from build123d import *

# Parameters (mm, degrees)
SKETCH1_W                                    = 250
SKETCH1_H                                    = 50
BOSS_EXTRUDE1_DEPTH                          = 20
FILLET1_R                                    = 10
LPATTERN1_COUNT                              = 3
LPATTERN1_PITCH                              = 60
CBORE_FOR_M10_HEXAGON_SOCKET_HEAD_CA_2_COUNT = 2
CBORE_FOR_M10_HEXAGON_SOCKET_HEAD_CA_2_PITCH = 210


with BuildPart() as part:
    # Sketch1 → Boss-Extrude1 (new body)
    with BuildSketch(Plane.XY):
        with Locations((-50, 0)):
            Rectangle(SKETCH1_W, SKETCH1_H)
    extrude(amount=BOSS_EXTRUDE1_DEPTH)

    # Fillet1
    fillet1_edges = [part.edges().sort_by_distance(p)[0] for p in [
        (-175, 25, 10),
        (75, 25, 10),
        (75, -25, 10),
        (-175, -25, 10),
    ]]
    fillet(fillet1_edges, radius=FILLET1_R)

    # Sketch2 → CBORE for M8 Hexagon socket head cap screws1 (revolve, cut)
    with BuildSketch(Plane(origin=(10, 0, 20), x_dir=(0, -1, 0), z_dir=(1, 0, 0))):
        Polygon((0, 0), (0, 24.953872786), (4.5, 22.25), (4.5, 9), (7.5, 9), (7.5, 0), align=None)
    cbore_for_m8_hexagon_socket_head_cap_scr = revolve(axis=Axis((10, 0, 26.35), (0, 0, -1)), mode=Mode.SUBTRACT)

    # LPattern1: CBORE for M8 Hexagon socket head cap screws1 ×3
    with Locations(*[(-i * LPATTERN1_PITCH, 0, 0) for i in range(1, LPATTERN1_COUNT)]):
        add(cbore_for_m8_hexagon_socket_head_cap_scr, mode=Mode.SUBTRACT)

    # Sketch4 → CBORE for M10 Hexagon socket head cap screws1 (revolve, cut)
    with BuildSketch(Plane.YZ.offset(55)):
        Polygon((0, 0), (0, 30.804733405), (5.5, 27.5), (5.5, 11), (9, 11), (9, 0.025), (9.025, 0), align=None)
    cbore_for_m10_hexagon_socket_head_cap_sc = revolve(axis=Axis((55, 0, -6.35), (0, 0, 1)), mode=Mode.SUBTRACT)

    # CBORE for M10 Hexagon socket head ca 2: CBORE for M10 Hexagon socket head cap screws1 ×2
    with Locations(*[(-i * CBORE_FOR_M10_HEXAGON_SOCKET_HEAD_CA_2_PITCH, 0, 0) for i in range(1, CBORE_FOR_M10_HEXAGON_SOCKET_HEAD_CA_2_COUNT)]):
        add(cbore_for_m10_hexagon_socket_head_cap_sc, mode=Mode.SUBTRACT)


solid = part.part
Check sheet for the modelled part. Datum: model origin and axes. Units: mm. A direction names the side the tool comes from. Coordinates: 2 decimals unless noted, no trailing zeros. Write each loop counter-clockwise with the first axis right and the second up, starting at its lowest first coordinate (ties: lowest second). Pieces come first, ordered by that corner, then holes. Notation, with made-up numbers: M 8.25,79 L 61.25,79 A21 ccw 61.25,95 Z; hole C 3,72.5 d1. An arc over 180 degrees is marked long. Answer as CSV lines item,"result".
Q1. Mould release check, pull along X, two halves, no side actions. Record for faces 4 (the face through (72.15, 21.99, 10.14)), 5 (the face through (-52, 25, 10)), 6 (the face through (-159, -4, 11)): released by +X, released by -X, zero draft, split by the parting line, or undercut.
Check result:
face 4,"released by +X"
face 5,"zero draft"
face 6,"undercut"
Q2. Set-up check for faces 1 (the face through (63.786, -1.951, 5.436)), 2 (the face through (49.547, -0.716, 15.437)), 3 (the face through (15, 0, 11)): record each of +Z, -Z, +X, -X, +Y, -Y from which the full face is reachable in a straight line by a thin tool's end or side.
Check result:
face 1,"-Z"
face 2,"+Z, -Z"
face 3,"+Z"
Q3. Cross-section at C-C (x = 55). Record the boundary of the cut face in (y, z) (3 decimals).
Check result:
outline,"M -25,0 L -9.025,0 L -9,0.025 L -9,11 L -5.5,11 L -5.5,20 L -25,20 Z; M 5.5,11 L 9,11 L 9,0.025 L 9.025,0 L 25,0 L 25,20 L 5.5,20 Z"
Q4. Cross-section at D-D (y = 0). Count the separate pieces of the cut face and the enclosed holes in it, then the cut area to 3 significant figures.
Check result:
separate pieces,"6"
enclosed holes,"0"
area,"3,700 mm^2"
Q5. Go/stop test with flat-tipped pins: pin 1 (2 mm diameter, centred on y = 20, z = 8.5, fed in from -X); pin 2 (4.5 mm diameter, centred on x = -46.5, y = 3, fed in from +Z); pin 3 (9 mm diameter, centred on x = 57.5, y = 1, fed in from -Z). Record where each tip stops, or that it passes through.
Check result:
pin 1,"x = -174.17"
pin 2,"z = 11"
pin 3,"z = 11"
Q6. Material ranges on probe 1 along X at (y, z) = (0, 14.5); probe 2 along X at (y, z) = (0, 5.5); probe 3 along Y at (x, z) = (-50, 16.25), recorded low to high. Write a range as from..to.
Check result:
probe 1,"-175..-160.5, -149.5..-117.5, -102.5..-57.5, -42.5..2.5, 17.5..49.5, 60.5..75"
probe 2,"-175..-164, -146..-114.5, -105.5..-54.5, -45.5..5.5, 14.5..46, 64..75"
probe 3,"-25..-7.5, 7.5..25"
Q7. Cross-section at B-B (z = 7.75). Record the boundary of the cut face in (x, y).
Check result:
outline,"M -175,-15 A10 ccw -165,-25 L 65,-25 A10 ccw 75,-15 L 75,15 A10 ccw 65,25 L -165,25 A10 ccw -175,15 Z; hole C -155,0 d18; hole C -110,0 d9; hole C -50,0 d9; hole C 10,0 d9; hole C 55,0 d18"
Q8. Cross-section at A-A (x = -50). Record the boundary of the cut face in (y, z), then the cut area to 3 significant figures.
Check result:
outline,"M -25,0 L -4.5,0 L -4.5,11 L -7.5,11 L -7.5,20 L -25,20 Z; M 4.5,0 L 25,0 L 25,20 L 7.5,20 L 7.5,11 L 4.5,11 Z"
area,"766 mm^2"
